Part model, mm, in its own coordinate system. A direction names the side the tool comes from. Coordinates: 2 decimals unless noted, no trailing zeros. Write each loop counter-clockwise with the first axis right and the second up, starting at its lowest first coordinate (ties: lowest second). Pieces come first, ordered by that corner, then holes. Notation, with made-up numbers: (51.5, 12) - (58.5, 12) arc R3 ccw to (58.5, 17) - close; hole circle Ø10 at (-13.5, 37.25). An arc over 180 degrees is marked (long way). Use one line per item in the form item = value. Start each with the question number.
from build123d import *

# Parameters (mm, degrees)
BRACKET_BODY_DEPTH          = 50
BASE_HOLES_8_SET_A_SKETCH_R = 4
BASE_HOLES_8_SET_A_DEPTH    = 100
STEP_NOTCH_SKETCH_W         = 60
STEP_NOTCH_SKETCH_H         = 42
STEP_NOTCH_DEPTH            = 15
WEB_BORE_18_SKETCH_R        = 9
WEB_BORE_18_DEPTH           = 100
BASE_HOLES_8_SET_B_SKETCH_R = 4
BASE_HOLES_8_SET_B_DEPTH    = 100
BASE_HOLES_6_SKETCH_R       = 3
BASE_HOLES_6_DEPTH          = 100


with BuildPart() as part:
    # Bracket Profile Sketch → Bracket Body (new, symmetric)
    with BuildSketch(Plane.XY):
        Polygon((0, 0), (-102.5, 0), (-102.5, 20), (-2.5, 20), (-2.5, 35), (57.5, 35), (57.5, 85), (77.5, 85), (77.5, 15), (102.5, 15), (102.5, 0), align=None)
    extrude(amount=BRACKET_BODY_DEPTH, both=True)

    # Base Holes Ø8 Set A Sketch → Base Holes Ø8 Set A (cut)
    with BuildSketch(Plane(origin=(0, 15, 0), x_dir=(1, 0, 0), z_dir=(0, 1, 0))):
        with Locations(Location((90.5, 35, 0), (0, 0, 180))):
            Circle(BASE_HOLES_8_SET_A_SKETCH_R)
        with Locations(Location((90.5, -35, 0), (0, 0, 180))):
            Circle(BASE_HOLES_8_SET_A_SKETCH_R)
    extrude(amount=-BASE_HOLES_8_SET_A_DEPTH, mode=Mode.SUBTRACT)

    # Step Notch Sketch → Step Notch (cut)
    with BuildSketch(Plane(origin=(0, 35, 0), x_dir=(1, 0, 0), z_dir=(0, 1, 0))):
        with Locations((27.5, 0)):
            Rectangle(STEP_NOTCH_SKETCH_W, STEP_NOTCH_SKETCH_H)
    extrude(amount=-STEP_NOTCH_DEPTH, mode=Mode.SUBTRACT)

    # Web Bore Ø18 Sketch → Web Bore Ø18 (cut)
    with BuildSketch(Plane(origin=(77.5, 0, 0), x_dir=(0, 0, -1), z_dir=(1, 0, 0))):
        with Locations((0, 45)):
            Circle(WEB_BORE_18_SKETCH_R)
    extrude(amount=-WEB_BORE_18_DEPTH, mode=Mode.SUBTRACT)

    # Base Holes Ø8 Set B Sketch → Base Holes Ø8 Set B (cut)
    with BuildSketch(Plane(origin=(0, 20, 0), x_dir=(1, 0, 0), z_dir=(0, 1, 0))):
        with Locations(Location((-20.5, -35, 0), (0, 0, 180))):
            Circle(BASE_HOLES_8_SET_B_SKETCH_R)
        with Locations(Location((-20.5, 35, 0), (0, 0, 180))):
            Circle(BASE_HOLES_8_SET_B_SKETCH_R)
    extrude(amount=-BASE_HOLES_8_SET_B_DEPTH, mode=Mode.SUBTRACT)

    # Base Holes Ø6 Sketch → Base Holes Ø6 (cut)
    with BuildSketch(Plane(origin=(0, 20, 0), x_dir=(1, 0, 0), z_dir=(0, 1, 0))):
        with Locations(Location((-80, -17, 0), (0, 0, 180))):
            Circle(BASE_HOLES_6_SKETCH_R)
        with Locations(Location((-80, 17, 0), (0, 0, 180))):
            Circle(BASE_HOLES_6_SKETCH_R)
    extrude(amount=-BASE_HOLES_6_DEPTH, mode=Mode.SUBTRACT)


solid = part.part
Q1. Slice it at B-B (y = 45). List the corners of the cut face in (x, z), plus the area to 3 significant figures.
Q2. Mould opens along X. For faces 3 (the cylindrical face through (-77.6, 10.1, 15.2)), 4 (the flat face through (77.5, 58, 1)), 5 (the flat face through (90, 15, 1)) say: released by +X, released by -X, zero draft, split by the parting line, or undercut.
Q3. Slice it at A-A (x = -80). List the corners of the cut face in (y, z), plus the area to 3 significant figures.
Q4. Pin check, flat tips, straight feed: P1, Ø12, axis at y = 27.5, z = 24.5, coming from the -X side; P2, Ø1, axis at x = 82, z = 3, coming from the +Y side; P3, Ø12, axis at y = 25.5, z = -2, coming from the +X side. Stop position of each tip, or through.
Q5. Slice it at C-C (z = -17). List the corners of the cut face in (x, y).
Q6. Slice it at D-D (z = 11.5). List the corners of the cut face in (x, y).
Q7. Which spindle directions (+Z, -Z, +X, -X, +Y, -Y) get a long thin tool onto all of the face, cutting with end or side? Do faces 1 (the flat face through (24, 24, 50)), 2 (the flat face through (-2.5, 27, 36)). Say none if no direction does.
Q8. Drill centre lines: probe 1 along Z at (x, y) = (-20, 15); probe 2 along Z at (x, y) = (22.5, 33); probe 3 along Y at (x, z) = (-3, -31.5). Where is each one in solid material? Low to high.
Solution:
q1.outline = (57.5, -50) - (77.5, -50) - (77.5, -9) - (57.5, -9) - close; (57.5, 9) - (77.5, 9) - (77.5, 50) - (57.5, 50) - close
q1.area = 1,640 mm2
q2.face_3 = undercut
q2.face_4 = released by +X
q2.face_5 = zero draft
q3.outline = (0, -50) - (20, -50) - (20, -20) - (0, -20) - close; (0, -14) - (20, -14) - (20, 14) - (0, 14) - close; (0, 20) - (20, 20) - (20, 50) - (0, 50) - close
q3.area = 1,760 mm2
q4.P1 = -2.5
q4.P2 = 15
q4.P3 = 77.5
q5.outline = (-102.5, 0) - (-83, 0) - (-83, 20) - (-102.5, 20) - close; (-77, 0) - (102.5, 0) - (102.5, 15) - (77.5, 15) - (77.5, 85) - (57.5, 85) - (57.5, 20) - (-77, 20) - close
q6.outline = (-102.5, 0) - (102.5, 0) - (102.5, 15) - (77.5, 15) - (77.5, 85) - (57.5, 85) - (57.5, 20) - (-102.5, 20) - close
q7.face_1 = +Z, +X, -X, +Y, -Y
q7.face_2 = +Z, -Z, -X, +Y
q8.probe_1 = -50 to -38.97, -31.03 to 31.03, 38.97 to 50
q8.probe_2 = -50 to -21, 21 to 50
q8.probe_3 = 0 to 20
